```python
from build123d import *

# Parameters (mm, degrees)
END_RIM_A_PROFILE_25_R       = 12.5
END_RIM_A_25_DEPTH           = 1.25
RUN_START                    = -2.5
RUN_TUBE_PROFILE_22_5_R      = 11.25
RUN_TUBE_22_5_DEPTH          = 45
END_RIM_B_PROFILE_25_R       = 12.5
END_RIM_B_25_DEPTH           = 2.5
RUN_BORE_PROFILE_20_R        = 10
RUN_BORE_20_DEPTH            = 54.033008589
RIM_FILLETS_R1_R             = 1
BRANCH_START                 = 26.25
BRANCH_RIM_25_DEPTH          = 2.5
BRANCH_TUBE_PROFILE_22_5_R   = 11.25
BRANCH_TUBE_22_5_DEPTH       = 27
RUN_BORE_CLEARANCE_PROFILE_R = 10
RUN_BORE_CLEARANCE_CUT_DEPTH = 60.015358255
BRANCH_BORE_20_REACH         = 67.072
BRANCH_BORE_20_END_RADIUS    = 10
BRANCH_BORE_PROFILE_20_R     = 10


with BuildPart() as part:
    # End Rim A Profile _25 → End Rim A _25 (new, symmetric)
    with BuildSketch(Plane.XY):
        Circle(END_RIM_A_PROFILE_25_R)
    extrude(amount=END_RIM_A_25_DEPTH, both=True)

    # Run Tube Profile _22.5 → Run Tube _22.5 (add)
    with BuildSketch(Plane.XY.offset(1.25).offset(RUN_START)):
        Circle(RUN_TUBE_PROFILE_22_5_R)
    extrude(amount=-RUN_TUBE_22_5_DEPTH)

    # End Rim B Profile _25 → End Rim B _25 (add)
    with BuildSketch(Plane(origin=(0, 0, -46.25), x_dir=(-1, 0, 0), z_dir=(0, 0, -1))):
        with Locations(Location((0, 0, 0), (0, 0, 180))):
            Circle(END_RIM_B_PROFILE_25_R)
    extrude(amount=END_RIM_B_25_DEPTH)

    # Run Bore Profile _20 → Run Bore _20 (cut, through all)
    with BuildSketch(Plane(origin=(0, 0, -48.75), x_dir=(-1, 0, 0), z_dir=(0, 0, -1))):
        Circle(RUN_BORE_PROFILE_20_R)
    extrude(amount=-RUN_BORE_20_DEPTH, mode=Mode.SUBTRACT)

    # Rim Fillets R1
    rim_fillets_r1_edges = [part.edges().sort_by_distance(p)[0] for p in [
        (-11.25, 0, -46.25),
        (-11.25, 0, -1.25),
    ]]
    fillet(rim_fillets_r1_edges, radius=RIM_FILLETS_R1_R)



with BuildPart() as body_2:
    # Branch Rim Profile _25 → Branch Rim _25 (new body)
    with BuildSketch(Plane(origin=(0, 0, 0), x_dir=(1, 0, 0), z_dir=(0, 1, 0)).offset(BRANCH_START)):
        with BuildLine():
            ThreePointArc((12.5, 23.75), (8.838834765, 32.588834765), (0, 36.25))
            Line((0, 36.25), (0, 11.25))
            ThreePointArc((0, 11.25), (8.838834765, 14.911165235), (12.5, 23.75))
        make_face()
        with BuildLine():
            Line((0, 11.25), (0, 36.25))
            ThreePointArc((0, 36.25), (-12.5, 23.75), (0, 11.25))
        make_face()
    extrude(amount=BRANCH_RIM_25_DEPTH)


with BuildPart() as part_1:
    add(part.part)

    add(body_2.part)  # Branch Tube _22.5 merges body 2
    # Branch Tube Profile _22.5 → Branch Tube _22.5 (add)
    with BuildSketch(Plane(origin=(0, 0, 0), x_dir=(1, 0, 0), z_dir=(0, 1, 0))):
        with Locations((0, 23.75)):
            Circle(BRANCH_TUBE_PROFILE_22_5_R)
    extrude(amount=BRANCH_TUBE_22_5_DEPTH)

    # Run Bore Clearance Profile → Run Bore Clearance Cut (cut, through all)
    with BuildSketch(Plane.XY.offset(1.25)):
        with Locations(Location((0, 0, 0), (0, 0, 180))):
            Circle(RUN_BORE_CLEARANCE_PROFILE_R)
    extrude(amount=-RUN_BORE_CLEARANCE_CUT_DEPTH, mode=Mode.SUBTRACT)

    # Branch Bore _20: up to this cylinder (the profile starts outside it)
    branch_bore_20_end = Plane(origin=(0, 0, -23.75), z_dir=(0, 0, -1)) * Cylinder(BRANCH_BORE_20_END_RADIUS, 155.144, mode=Mode.PRIVATE)
    # Branch Bore Profile _20 → Branch Bore _20 (cut, up to the surface)
    with BuildSketch(Plane(origin=(0, 28.75, 0), x_dir=(1, 0, 0), z_dir=(0, 1, 0)), mode=Mode.PRIVATE) as branch_bore_20_sk1:
        with Locations(Location((0, 23.75, 0), (0, 0, 270))):
            Circle(BRANCH_BORE_PROFILE_20_R)
    branch_bore_20_tool1 = extrude(branch_bore_20_sk1.sketch, amount=-BRANCH_BORE_20_REACH, mode=Mode.PRIVATE) - branch_bore_20_end
    add(branch_bore_20_tool1.solids().sort_by_distance((0, 28.75, -23.75))[0], mode=Mode.SUBTRACT)


solid = part_1.part
```
For this review, take the finished solid that the model builds, in its own axes (mm). A direction names the side the tool comes from. Round coordinates to 2 decimals unless told otherwise and drop trailing zeros. Write each loop counter-clockwise with the first axis right and the second up, starting at its lowest first coordinate (ties: lowest second). Pieces come first, ordered by that corner, then holes. Notation, with made-up numbers: M 25.5,69.5 L 79.5,69.5 A24 ccw 79.5,104.5 Z; hole C 82,1 d8. An arc over 180 degrees is marked long. One line per item, written item: value. Start each with the question number.
(1) We need section A-A (y = 13.5). Give the boundary of the cut face in (x, z), and give its area (3 significant figures).
(2) We need section C-C (z = -40). Give the boundary of the cut face in (x, y), and give its area (3 significant figures).
(3) Machinability: for faces 1 (the flat face through (-5, 26.25, -34)), 2 (the flat face through (-6, 28.75, -32)), 3 (the cylindrical face through (11.923, 3.755, 0.018)), which of the approach directions +Z, -Z, +X, -X, +Y, -Y give a long, thin tool a straight path to every point of the face, cutting with its end or side? Answer none if there is none.
(4) Wall thickness on line 1 (X direction, y = 0, z = -20); line 2 (X direction, y = -7, z = -29); line 3 (Y direction, x = 6.25, z = -39): over which ranges is each line inside the solid? List them lowest first.
(5) The part is to be moulded in two halves that separate along Z. For faces 4 (the flat face through (-0.1, 10.2, 1.25)), 5 (the cylindrical face through (0.44, 17.77, -33.74)), 6 (the cylindrical face through (11.923, -3.755, -47.482)), say which applies: released by +Z, released by -Z, zero draft, split by the parting line, or undercut.
(6) We need section D-D (x = -1.25). Count the separate pieces of the cut face and the enclosed holes in it, and give its area (3 significant figures).
(7) We need section B-B (z = -18). Give the boundary of the cut face in (x, y).
(8) Insertion check: pin 1 (1 mm diameter, centred on x = 1.5, z = -40.5, fed in from -Y); pin 2 (4 mm diameter, centred on x = -8, y = 19.5, fed in from -Z); pin 3 (7.5 mm diameter, centred on x = 2, y = -3.5, fed in from +Z); pin 4 (1.5 mm diameter, centred on x = 4.5, z = -21.5, fed in from +Y). Each pin has a flat end and moves straight along its axis. Give the tip position at first contact, or say it passes through.
Result:
1. outline: C 0,-23.75 d22.5; hole C 0,-23.75 d20
1. area: 83.4 mm²
2. outline: C 0,0 d22.5; hole C 0,0 d20
2. area: 83.4 mm²
3. face 1: none
3. face 2: +Z, -Z, +X, -X, +Y
3. face 3: +Z
4. line 1: -11.25 to -10, 10 to 11.25
4. line 2: -8.81 to -7.14, 7.14 to 8.81
4. line 3: -9.35 to -7.81, 7.81 to 9.35
5. face 4: released by +Z
5. face 5: undercut
5. face 6: zero draft
6. separate pieces: 3
6. enclosed holes: 0
6. area: 165 mm²
7. outline: M -11.1,26.25 L -9.67,26.25 L -9.67,5.75 A11.25 ccw long 9.67,5.75 L 9.67,26.25 L 11.1,26.25 L 11.1,28.75 L 8.18,28.75 L 8.18,5.75 A10 cw long -8.18,5.75 L -8.18,28.75 L -11.1,28.75 Z
8. pin 1: y = -11.21
8. pin 2: z = -33.27
8. pin 3: through
8. pin 4: y = -8.51
